```python
from build123d import *

# Parameters (mm, degrees)
SKETCH_1_W          = 150
SKETCH_1_H          = 100
EXTRUDE_1_DEPTH     = 10
HOLE_WIZARD_M12_1_D = 10.2
CUT_EXTRUDE_1_DEPTH = 91.691785736
CHAMFER_1_SIZE      = 5


with BuildPart() as part:
    # 草图1 → 凸台-拉伸1 (new body)
    with BuildSketch(Plane(origin=(0, 0, 0), x_dir=(0, 0, -1), z_dir=(1, 0, 0))):
        Rectangle(SKETCH_1_W, SKETCH_1_H)
    extrude(amount=EXTRUDE_1_DEPTH)

    # M12 螺纹孔1 (through all)
    with Locations(Plane(origin=(10, 0, 0), x_dir=(0, 0, -1), z_dir=(1, 0, 0))):
        with Locations((-28.284271247, 28.284271247), (28.284271247, 28.284271247), (28.284271247, -28.284271247), (-28.284271247, -28.284271247)):
            Hole(HOLE_WIZARD_M12_1_D / 2)

    # 草图4 → 切除-拉伸1 (cut, through all)
    with BuildSketch(Plane(origin=(10, 0, 0), x_dir=(0, 0, -1), z_dir=(1, 0, 0))):
        with BuildLine():
            Line((-53.75, 40), (-53.75, 10))
            ThreePointArc((-53.75, 10), (-60, 3.75), (-66.25, 10))
            Line((-66.25, 10), (-66.25, 40))
            ThreePointArc((-66.25, 40), (-60, 46.25), (-53.75, 40))
        make_face()
        with BuildLine():
            Line((53.75, 40), (53.75, 10))
            ThreePointArc((53.75, 10), (60, 3.75), (66.25, 10))
            Line((66.25, 10), (66.25, 40))
            ThreePointArc((66.25, 40), (60, 46.25), (53.75, 40))
        make_face()
        with BuildLine():
            Line((-53.75, -40), (-53.75, -10))
            ThreePointArc((-53.75, -10), (-60, -3.75), (-66.25, -10))
            Line((-66.25, -10), (-66.25, -40))
            ThreePointArc((-66.25, -40), (-60, -46.25), (-53.75, -40))
        make_face()
        with BuildLine():
            Line((53.75, -40), (53.75, -10))
            ThreePointArc((53.75, -10), (60, -3.75), (66.25, -10))
            Line((66.25, -10), (66.25, -40))
            ThreePointArc((66.25, -40), (60, -46.25), (53.75, -40))
        make_face()
    extrude(amount=-CUT_EXTRUDE_1_DEPTH, mode=Mode.SUBTRACT)

    # 倒角1
    chamfer_1_edges = [part.edges().sort_by_distance(p)[0] for p in [
        (5, -50, -75),
        (5, -50, 75),
        (5, 50, 75),
        (5, 50, -75),
    ]]
    chamfer(chamfer_1_edges, length=CHAMFER_1_SIZE)


solid = part.part
```
The listing builds one solid part. Answer for the finished solid, in the listing's coordinates (mm). A direction names the side the tool comes from. Round coordinates to 2 decimals unless told otherwise and drop trailing zeros. Loops run counter-clockwise (first coordinate to the right, second up) from the corner with the lowest first, then second, coordinate; pieces in that order, holes last.
Q1. Which of the six approach directions +Z, -Z, +X, -X, +Y, -Y give full straight-line access (tool end or side, diameter ignored) to faces 1 (the face through (5, 48, 72)), 2 (the face through (5, 25, -66.25))?
Q2. For a pull along Y with two mould halves and no side action, classify faces 3 (the face through (5.07, 46.25, 60.14)), 4 (the face through (5, -1, 75)), 5 (the face through (5, -25, 53.75)), 6 (the face through (5, -48, 72)) as released by +Y, released by -Y, zero draft, split by the parting line, or undercut.
Q3. Section A-A, the plane y = -14.5 is taken. Determine the outline of the cut face in (x, z), then the cut area to 3 significant figures.
Q4. Find the intervals of material crossed by line 1 (Y direction, x = 4.5, z = -28); line 2 (Z direction, x = 3.5, y = -22); line 3 (Y direction, x = 5.75, z = -60.5), in increasing order.
Q5. Section C-C, the plane x = 5.5 is taken. Count the separate pieces of the cut face and the enclosed holes in it, then the cut area to 3 significant figures.
Q6. Section B-B, the plane z = 60 is taken. Determine the outline of the cut face in (x, y), then the cut area to 3 significant figures.
Completed:
1. face 1: +Z, +X, -X, +Y
1. face 2: +X, -X
2. face 3: undercut
2. face 4: zero draft
2. face 5: undercut
2. face 6: released by -Y
3. outline: (0, -75) - (10, -75) - (10, -66.25) - (0, -66.25) - close; (0, -53.75) - (10, -53.75) - (10, 53.75) - (0, 53.75) - close; (0, 66.25) - (10, 66.25) - (10, 75) - (0, 75) - close
3. area: 1,250 mm2
4. line 1: y = -50 to -33.38, -23.19 to 23.19, 33.38 to 50
4. line 2: z = -75 to -66.25, -53.75 to 53.75, 66.25 to 75
4. line 3: y = -50 to -46.23, -3.77 to 3.77, 46.23 to 50
5. separate pieces: 1
5. enclosed holes: 8
5. area: 12,600 mm2
6. outline: (0, -50) - (10, -50) - (10, -46.25) - (0, -46.25) - close; (0, -3.75) - (10, -3.75) - (10, 3.75) - (0, 3.75) - close; (0, 46.25) - (10, 46.25) - (10, 50) - (0, 50) - close
6. area: 150 mm2
